```python
from build123d import *

# Parameters (mm, degrees)
BOSS_EXTRUDE1_DEPTH = 5
CHAMFER1_SIZE       = 25


with BuildPart() as part:
    # Sketch1 → Boss-Extrude1 (new, symmetric)
    with BuildSketch(Plane.XY):
        Polygon((0, 0), (110, 0), (110, 30), (15, 180), (0, 180), align=None)
    extrude(amount=BOSS_EXTRUDE1_DEPTH, both=True)

    # Chamfer1
    chamfer1_edges = [part.edges().sort_by_distance(p)[0] for p in [
        (0, 0, 0),
    ]]
    chamfer(chamfer1_edges, length=CHAMFER1_SIZE)


solid = part.part
```
Part model, mm, in its own coordinate system. Give positions to 0.01 mm unless a question says otherwise; leave off trailing zeros. Loops run counter-clockwise (first coordinate to the right, second up) from the corner with the lowest first, then second, coordinate; pieces in that order, holes last. Notation, with made-up numbers: M 59.5,82.25 L 71.5,82.25 A25 ccw 71.5,115.25 Z; hole C 53,7 d3. An arc over 180 degrees is marked long. Return JSON: item names as keys, results as strings.
1) Drill centre lines: line 1 (Y direction, x = 10, z = 3.5); line 2 (X direction, y = 39.5, z = -0.25); line 3 (X direction, y = 63, z = 0.5). Where is each one in solid material? Low to high.
Calculated:
{"line 1": "y = 15 to 180", "line 2": "x = 0 to 103.98", "line 3": "x = 0 to 89.1"}
2) Saw through at C-C, the plane y = 66. List the corners of the cut face in (x, z), then the cut area to 3 significant figures.
Calculated:
{"outline": "M 0,-5 L 87.2,-5 L 87.2,5 L 0,5 Z", "area": "872 mm2"}
3) Pull direction X, two halves, no side cores. Call faces 1 (the face through (42, 71, -5)), 2 (the face through (63.165, 103.95, 0.07)), 3 (the face through (0, 104, 0)): released by +X, released by -X, zero draft, split by the parting line, or undercut.
Calculated:
{"face 1": "zero draft", "face 2": "released by +X", "face 3": "released by -X"}
4) Saw through at A-A, the plane z = 0.5. List the corners of the cut face in (x, y).
Calculated:
{"outline": "M 0,25 L 25,0 L 110,0 L 110,30 L 15,180 L 0,180 Z"}
5) Flat gauge pins, fed straight in: pin 1 Ø4 at (x, z) = (89, -4) entering from +Y; pin 2 Ø4 at (x, z) = (57, -3) entering from +Y; pin 3 Ø3 at (x, z) = (56, 0) entering from +Y. Where does each tip first touch, or does it go through?
Calculated:
{"pin 1": "stops at y = 66.32", "pin 2": "stops at y = 116.84", "pin 3": "stops at y = 117.63"}
6) Saw through at B-B, the plane x = 7. List the corners of the cut face in (y, z), then the cut area to 3 significant figures.
Calculated:
{"outline": "M 18,-5 L 180,-5 L 180,5 L 18,5 Z", "area": "1,620 mm2"}
